Verification items for the finished model (mm, model axes). A direction names the side the tool comes from. Round coordinates to 2 decimals unless told otherwise and drop trailing zeros. Order: outer loops, then holes, each group sorted by start corner. A loop starts at its lowest first (then second) coordinate and runs counter-clockwise, first axis right, second up. Notation, with made-up numbers: M -27.5,82.25 L -7.5,82.25 A34 ccw -7.5,113.25 Z; hole C 86,-14 d11. An arc over 180 degrees is marked long. Answer as a JSON object with one key per item and string values. Group by question number.
```python
from build123d import *

# Parameters (mm, degrees)
SKETCH1_R           = 11.25
SKETCH1_R_2         = 2
BOSS_EXTRUDE1_DEPTH = 5
SKETCH2_R           = 4
SKETCH2_R_2         = 2
BOSS_EXTRUDE2_DEPTH = 4
CUT_EXTRUDE1_DEPTH  = 10


with BuildPart() as part:
    # Sketch1 → Boss-Extrude1 (new body)
    with BuildSketch(Plane.XY):
        Circle(SKETCH1_R)
        with Locations((0, 8)):
            Circle(SKETCH1_R_2, mode=Mode.SUBTRACT)
        with Locations((8, 0)):
            Circle(SKETCH1_R_2, mode=Mode.SUBTRACT)
        with Locations((0, -8)):
            Circle(SKETCH1_R_2, mode=Mode.SUBTRACT)
        with Locations((-8, 0)):
            Circle(SKETCH1_R_2, mode=Mode.SUBTRACT)
        Circle(SKETCH1_R_2, mode=Mode.SUBTRACT)
    extrude(amount=BOSS_EXTRUDE1_DEPTH)

    # Sketch2 → Boss-Extrude2 (add)
    with BuildSketch(Plane.XY.offset(5)):
        Circle(SKETCH2_R)
        Circle(SKETCH2_R_2, mode=Mode.SUBTRACT)
    extrude(amount=BOSS_EXTRUDE2_DEPTH)

    # Sketch4 → Cut-Extrude1 (cut)
    with BuildSketch(Plane(origin=(7.954951288, -7.954951288, 0), x_dir=(-0.7071067811865475, -0.7071067811865477, 0), z_dir=(0.7071067811865477, -0.7071067811865475, 0))):
        with BuildLine():
            ThreePointArc((1.5, -2.45834938), (1.060660172, -1.397689208), (0, -0.95834938))
            Line((0, -0.95834938), (0, -3.95834938))
            ThreePointArc((0, -3.95834938), (1.060660172, -3.519009552), (1.5, -2.45834938))
        make_face()
        with BuildLine():
            Line((0, -3.95834938), (0, -0.95834938))
            ThreePointArc((0, -0.95834938), (-1.5, -2.45834938), (0, -3.95834938))
        make_face()
    extrude(amount=-CUT_EXTRUDE1_DEPTH, mode=Mode.SUBTRACT)


solid = part.part
```
Q1. Release check for a two-part mould opening along X. For faces 1 (the face through (-2, -1, 9)), 2 (the face through (-9.6, -1.2, 2.5)), 3 (the face through (-0.867, -3.905, 6.972)) record: released by +X, released by -X, zero draft, split by the parting line, or undercut.
Q2. Thickness scan on line 1 (Y direction, x = 0, z = 3.95); line 2 (Y direction, x = 1.75, z = 3.5); line 3 (X direction, y = -1, z = 3.5). Record the ranges inside material, lowest first. Write a range as from..to.
Q3. Tool access check on faces 4 (the face through (-1.474, 1.352, 4.437)), 5 (the face through (5, 0, 5)). Record the directions out of +Z, -Z, +X, -X, +Y, -Y that give a thin tool (end or side, any length) a straight path to the whole face; none if there is none.
Q4. Gauge pin test, flat ends, axial feed: pin 1 Ø1.5 at (y, z) = (3.5, 7.5) entering from +X; pin 2 Ø4 at (x, y) = (0, -6.5) entering from +Z; pin 3 Ø3.5 at (x, y) = (-8, 0) entering from +Z; pin 4 Ø1.5 at (x, z) = (-2.5, 1) entering from -Y. Record the tip position at first contact, or that the pin passes through.
Q5. Cross-section at A-A, the plane y = 8. Record the cut outline in (x, z), then the cut area to 3 significant figures.
Conclusion:
{
 "1": {"face 1": "zero draft", "face 2": "undercut", "face 3": "split by the parting line"},
 "2": {"line 1": "-11.25..-10, -6..-2, 2..6, 10..11.25", "line 2": "-11.11..-8.97, -7.03..-3.28, 0.97..7.03, 8.97..11.11", "line 3": "-11.21..-9.73, -6.27..-1.73, 2.53..6.27, 9.73..11.21"},
 "3": {"face 4": "+Z, -Z", "face 5": "+Z"},
 "4": {"pin 1": "x = 2.9", "pin 2": "z = 5", "pin 3": "through", "pin 4": "y = -11.11"},
 "5": {"outline": "M -7.91,0 L -2,0 L -2,5 L -7.91,5 Z; M 2,0 L 7.91,0 L 7.91,5 L 2,5 Z", "area": "59.1 mm2"}
}
